```python
from build123d import *

# Parameters (mm, degrees)
SKETCH_1_W      = 66
SKETCH_1_H      = 66
SKETCH_1_W_2    = 51
SKETCH_1_H_2    = 51
EXTRUDE_1_DEPTH = 30


with BuildPart() as part:
    # 草图1 → 凸台-拉伸1 (new, symmetric)
    with BuildSketch(Plane.XY):
        Rectangle(SKETCH_1_W, SKETCH_1_H)
        Rectangle(SKETCH_1_W_2, SKETCH_1_H_2, mode=Mode.SUBTRACT)
    extrude(amount=EXTRUDE_1_DEPTH, both=True)


solid = part.part
```
For this review, take the finished solid that the model builds, in its own axes (mm). A direction names the side the tool comes from. Coordinates: 2 decimals unless noted, no trailing zeros. Loops run counter-clockwise (first coordinate to the right, second up) from the corner with the lowest first, then second, coordinate; pieces in that order, holes last.
1. Mouldability with a two-part tool opening along Y and no side actions: class faces 3 (the flat face through (0, 33, 0)), 4 (the flat face through (0, -33, 0)), 5 (the flat face through (0, 25.5, 0)) as +Y half, -Y half, draft (parallel to the pull), parting line (faces both ways), or undercut.
2. Add section A-A, the plane y = 16. Give the boundary of the cut face in (x, z), then the cut area to 3 significant figures.
3. Add section B-B, the plane z = -1.5. Give the boundary of the cut face in (x, y).
4. For line 1 (Y direction, x = 14.5, z = -24.5), list the stretches that pass through material, from the lowest coordinate up.
5. For faces 1 (the flat face through (-33, 0, 0)), 2 (the flat face through (-25.5, 0, 0)), list the 3-axis set-ups (+Z, -Z, +X, -X, +Y, -Y) from which the entire face can be reached by the end or side of a thin tool; tool diameter is ignored.
Result:
1. face 3: +Y half
1. face 4: -Y half
1. face 5: undercut
2. outline: (-33, -30) - (-25.5, -30) - (-25.5, 30) - (-33, 30) - close; (25.5, -30) - (33, -30) - (33, 30) - (25.5, 30) - close
2. area: 900 mm2
3. outline: (-33, -33) - (33, -33) - (33, 33) - (-33, 33) - close; hole (-25.5, -25.5) - (25.5, -25.5) - (25.5, 25.5) - (-25.5, 25.5) - close
4. line 1: y = -33 to -25.5, 25.5 to 33
5. face 1: +Z, -Z, -X, +Y, -Y
5. face 2: +Z, -Z
